from build123d import *

# Parameters (mm, degrees)
BASE_BLOCK_SKETCH_W   = 13
BASE_BLOCK_SKETCH_H   = 50
BASE_BLOCK_DEPTH      = 75
BASE_END_ROUND_R25_R  = 25
BASE_EDGE_FILLET_R6_R = 6
ARM_WEB_DEPTH         = 35
HUB_BOSS_SKETCH_R     = 19
HUB_BOSS_SKETCH_R_2   = 6.5
HUB_BOSS_DEPTH        = 30
UPPER_LUG_DEPTH       = 8
CURVED_START          = -20
CURVED_BLADE_DEPTH    = 20
LUG_FILLET_R6_A_R     = 6
LUG_FILLET_R6_B_R     = 6


with BuildPart() as part:
    # Base Block Sketch → Base Block (new body)
    with BuildSketch(Plane.XY):
        with Locations((6.5, 25)):
            Rectangle(BASE_BLOCK_SKETCH_W, BASE_BLOCK_SKETCH_H)
    extrude(amount=-BASE_BLOCK_DEPTH)

    # Base End Round R25
    base_end_round_r25_edges = [part.edges().sort_by_distance(p)[0] for p in [
        (6.5, 0, 0),
        (6.5, 0, -75),
    ]]
    fillet(base_end_round_r25_edges, radius=BASE_END_ROUND_R25_R)

    # Base Edge Fillet R6
    base_edge_fillet_r6_edges = [part.edges().sort_by_distance(p)[0] for p in [
        (6.5, 50, -75),
        (6.5, 50, 0),
    ]]
    fillet(base_edge_fillet_r6_edges, radius=BASE_EDGE_FILLET_R6_R)

    # Arm Web Sketch → Arm Web (add)
    with BuildSketch(Plane(origin=(0, 50, 0), x_dir=(1, 0, 0), z_dir=(0, 1, 0))):
        with BuildLine():
            Line((3, 62.41287987), (0, 62.41287987))
            Line((0, 62.41287987), (0, 37.41287987))
            Line((0, 37.41287987), (0, 12.41287987))
            Line((0, 12.41287987), (3, 12.41287987))
            ThreePointArc((3, 12.41287987), (10.583426132, 37.41287987), (3, 62.41287987))
        make_face()
    extrude(amount=ARM_WEB_DEPTH)



with BuildPart() as body_2:
    # Hub Boss Sketch → Hub Boss (new body)
    with BuildSketch(Plane(origin=(0, 30, 0), x_dir=(1, 0, 0), z_dir=(0, 1, 0))):
        with Locations(Location((85, 37.41287987, 0), (0, 0, 270))):
            Circle(HUB_BOSS_SKETCH_R)
        with Locations(Location((85, 37.41287987, 0), (0, 0, 270))):
            Circle(HUB_BOSS_SKETCH_R_2, mode=Mode.SUBTRACT)
    extrude(amount=HUB_BOSS_DEPTH)


with BuildPart() as part_1:
    add(part.part)

    add(body_2.part)  # Upper Lug merges body 2
    # Upper Lug Sketch → Upper Lug (add)
    with BuildSketch(Plane(origin=(0, 50, 0), x_dir=(1, 0, 0), z_dir=(0, 1, 0))):
        with BuildLine():
            Line((85, 56.41287987), (13, 56.41287987))
            Line((13, 56.41287987), (13, 18.41287987))
            Line((13, 18.41287987), (85, 18.41287987))
            ThreePointArc((85, 18.41287987), (66, 37.41287987), (85, 56.41287987))
        make_face()
    extrude(amount=-UPPER_LUG_DEPTH)

    # Curved Blade Sketch → Curved Blade (add)
    with BuildSketch(Plane(origin=(0, 50, 0), x_dir=(1, 0, 0), z_dir=(0, 1, 0)).offset(CURVED_START)):
        with BuildLine():
            Line((0, 34.91287987), (66.165191798, 34.91287987))
            ThreePointArc((66.165191798, 34.91287987), (66, 37.41287987), (66.165191798, 39.91287987))
            Line((66.165191798, 39.91287987), (0, 39.91287987))
            Line((0, 39.91287987), (0, 34.91287987))
        make_face()
    extrude(amount=CURVED_BLADE_DEPTH)

    # Lug Fillet R6 A
    lug_fillet_r6_a_edges = [part_1.edges().sort_by_distance(p)[0] for p in [
        (13, 46, -18.41287987),
    ]]
    fillet(lug_fillet_r6_a_edges, radius=LUG_FILLET_R6_A_R)

    # Lug Fillet R6 B
    lug_fillet_r6_b_edges = [part_1.edges().sort_by_distance(p)[0] for p in [
        (13, 46, -56.41287987),
    ]]
    fillet(lug_fillet_r6_b_edges, radius=LUG_FILLET_R6_B_R)


solid = part_1.part
Work out the finished part from the listing and answer in its coordinate system (mm). A direction names the side the tool comes from. Give positions to 0.01 mm unless a question says otherwise; leave off trailing zeros. Loops run counter-clockwise (first coordinate to the right, second up) from the corner with the lowest first, then second, coordinate; pieces in that order, holes last. Notation, with made-up numbers: (23.5, 59.5) -> (49.5, 59.5) arc R25 cw to (49.5, 91.5) -> close; hole circle Ø2 at (0, 60). An arc over 180 degrees is marked (long way). Use a Markdown table: item, result. Add a question column.
1. Section D-D on y = 69 is taken. Determine the outline of the cut face in (x, z).
2. For faces 1 (the flat face through (52, 46, -56.413)), 2 (the flat face through (2, 67, -62.413)), 3 (the cylindrical face through (10.58, 67.26, -37.04)), determine the directions among +Z, -Z, +X, -X, +Y, -Y from which every point of the face is accessible in a straight line to the end or side of a thin tool.
3. Section A-A on y = 38 is taken. Determine the outline of the cut face in (x, z), and give its area (3 significant figures).
4. Flat-ended cylindrical pins translate along their axes: pin 1 Ø1.5 at (x, y) = (1.5, 66) entering from -Z; pin 2 Ø9.5 at (x, y) = (34.5, 37) entering from -Z; pin 3 Ø3.5 at (x, y) = (26.5, 37.5) entering from +Z. Find the tip coordinate at first contact, or state that the pin passes through.
5. Determine the mould class of faces 4 (the flat face through (0, 42, -37)), 5 (the flat face through (40, 42, -26)), 6 (the cylindrical face through (6.591, 48.196, -73.289)), 7 (the cylindrical face through (14.8, 45.9, -16.7)) for opening direction X: released by +X, released by -X, zero draft, split by the parting line, or undercut.
6. Find the intervals of material crossed by probe 1 along Z at (x, y) = (84.5, 32); probe 2 along X at (y, z) = (28, -68); probe 3 along X at (y, z) = (56.5, -53), in increasing order.
7. Section C-C on z = -38 is taken. Determine the outline of the cut face in (x, y), and give its area (3 significant figures).
8. Section B-B on x = 35 is taken. Determine the outline of the cut face in (y, z), and give its area (3 significant figures).
Results below:
| question | item | result |
|---|---|---|
| 1 | outline | (0, -62.41) -> (3, -62.41) arc R45 ccw to (3, -12.41) -> (0, -12.41) -> close |
| 2 | face 1 | -Z, +X, +Y, -Y |
| 2 | face 2 | -Z, +X, -X, +Y |
| 2 | face 3 | +Y |
| 3 | outline | (0, -75) -> (13, -75) -> (13, -39.91) -> (66.17, -39.91) arc R19 ccw (long way) to (66.17, -34.91) -> (13, -34.91) -> (13, 0) -> (0, 0) -> close; hole circle Ø13 at (85, -37.41) |
| 3 | area | 2,240 mm^2 |
| 4 | pin 1 | stops at z = -62.41 |
| 4 | pin 2 | stops at z = -39.91 |
| 4 | pin 3 | stops at z = -34.91 |
| 5 | face 4 | released by -X |
| 5 | face 5 | undercut |
| 5 | face 6 | zero draft |
| 5 | face 7 | released by +X |
| 6 | probe 1 | z = -56.41 to -43.89, -30.93 to -18.42 |
| 6 | probe 2 | x = 0 to 13 |
| 6 | probe 3 | x = 0 to 7.8, 74.14 to 95.86 |
| 7 | outline | (0, 0) -> (13, 0) -> (13, 30) -> (78.53, 30) -> (78.53, 60) -> (66.01, 60) -> (66.01, 50) -> (10.58, 50) -> (10.58, 85) -> (0, 85) -> close; (91.47, 30) -> (103.99, 30) -> (103.99, 60) -> (91.47, 60) -> close |
| 7 | area | 2,830 mm^2 |
| 8 | outline | (30, -39.91) -> (42, -39.91) -> (42, -56.41) -> (50, -56.41) -> (50, -18.41) -> (42, -18.41) -> (42, -34.91) -> (30, -34.91) -> close |
| 8 | area | 364 mm^2 |
